```python
from build123d import *

# Parameters (mm, degrees)
SKETCH_1_W                   = 75
SKETCH_1_H                   = 65
EXTRUDE_1_DEPTH              = 7.5
HOLE_WIZARD_M4_1_D           = 4.5
HOLE_WIZARD_M4_1_CBORE_D     = 8
HOLE_WIZARD_M4_1_CBORE_DEPTH = 4.4
HOLE_WIZARD_8_0_8_1_D        = 8
HOLE_WIZARD_1_D              = 4.5
HOLE_WIZARD_1_CBORE_D        = 10
HOLE_WIZARD_1_CBORE_DEPTH    = 7.5
SKETCH_8_R                   = 4
CUT_EXTRUDE_1_DEPTH          = 4.5
CHAMFER_1_SIZE               = 4
SKETCH_9_W                   = 30
SKETCH_9_H                   = 12
CUT_EXTRUDE_2_DEPTH          = 52.841103383
HOLE_WIZARD_M4_1_2_D         = 3.3
FILLET_1_R                   = 3


with BuildPart() as part:
    # 草图1 → 凸台-拉伸1 (new, symmetric)
    with BuildSketch(Plane.XY):
        Rectangle(SKETCH_1_W, SKETCH_1_H)
    extrude(amount=EXTRUDE_1_DEPTH, both=True)

    # Hole Wizard M4 _1 (through all)
    with Locations(Plane.XY.offset(7.5)):
        with Locations((14.5, 1.75), (14.5, -13.75), (30, 1.75), (30, -13.75)):
            CounterBoreHole(HOLE_WIZARD_M4_1_D / 2, HOLE_WIZARD_M4_1_CBORE_D / 2, HOLE_WIZARD_M4_1_CBORE_DEPTH)

    # Ø8.0 (8) 直径孔1 (through all)
    with Locations(Plane.XY.offset(7.5)):
        with Locations((-17.5, 22.5), (-30, -22.5), (-5, -22.5)):
            Hole(HOLE_WIZARD_8_0_8_1_D / 2)

    # 孔1 (through all)
    with Locations(Plane.XY.offset(7.5)):
        with Locations((-17.5, 0), (-17.5, -12.5)):
            CounterBoreHole(HOLE_WIZARD_1_D / 2, HOLE_WIZARD_1_CBORE_D / 2, HOLE_WIZARD_1_CBORE_DEPTH)

    # 草图8 → 切除-拉伸1 (cut)
    with BuildSketch(Plane(origin=(0, 0, -7.5), x_dir=(-1, 0, 0), z_dir=(0, 0, -1))):
        with Locations((17.5, 0)):
            Circle(SKETCH_8_R)
        with Locations((17.5, -12.5)):
            Circle(SKETCH_8_R)
    extrude(amount=-CUT_EXTRUDE_1_DEPTH, mode=Mode.SUBTRACT)

    # 倒角1
    chamfer_1_edges = [part.edges().sort_by_distance(p)[0] for p in [
        (37.5, -32.5, 0),
        (-37.5, -32.5, 0),
        (-37.5, 32.5, 0),
        (37.5, 32.5, 0),
    ]]
    chamfer(chamfer_1_edges, length=CHAMFER_1_SIZE)

    # 草图9 → 切除-拉伸2 (cut, through all)
    with BuildSketch(Plane(origin=(0, 0, -7.5), x_dir=(-1, 0, 0), z_dir=(0, 0, -1))):
        with Locations((-17.5, 13.5)):
            Rectangle(SKETCH_9_W, SKETCH_9_H)
    extrude(amount=-CUT_EXTRUDE_2_DEPTH, mode=Mode.SUBTRACT)

    # Hole Wizard M4 _1 2 (through all)
    with Locations(Plane(origin=(0, 0, -7.5), x_dir=(-1, 0, 0), z_dir=(0, 0, -1))):
        with Locations((-17.5, 24)):
            Hole(HOLE_WIZARD_M4_1_2_D / 2)

    # 圆角1
    fillet_1_edges = [part.edges().sort_by_distance(p)[0] for p in [
        (2.5, 19.5, 0),
        (2.5, 7.5, 0),
        (32.5, 7.5, 0),
        (32.5, 19.5, 0),
    ]]
    fillet(fillet_1_edges, radius=FILLET_1_R)


solid = part.part
```
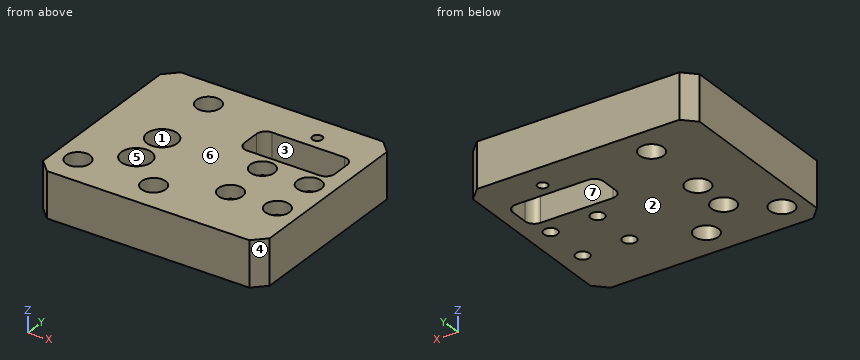
The model under review builds one solid part; all positions refer to its coordinate system, in mm. Face numbers are marked on the shaded views. A direction names the side the tool comes from. Round coordinates to 2 decimals unless told otherwise and drop trailing zeros. Order: outer loops, then holes, each group sorted by start corner. A loop starts at its lowest first (then second) coordinate and runs counter-clockwise, first axis right, second up.
(1) Take a section at B-B, the plane x = -5. State the section outline as (y, z) points, plus the area to 3 significant figures.
Working result:
outline: (-32.5, -7.5) - (-26.5, -7.5) - (-26.5, 7.5) - (-32.5, 7.5) - close; (-18.5, -7.5) - (32.5, -7.5) - (32.5, 7.5) - (-18.5, 7.5) - close
area: 855 mm2
(2) For P1, Ø4, axis at x = 15, y = -13, coming from the +Z side, flat-tipped, find the tip position at first contact; note if it passes through.
Working result:
P1: stops at z = 3.1
(3) Mouldability with a two-part tool opening along X and no side actions: class the marked faces 1, 2, 3 and 4 as released by +X, released by -X, zero draft, split by the parting line, or undercut.
Working result:
face 1: undercut
face 2: zero draft
face 3: undercut
face 4: released by +X
(4) Take a section at A-A, the plane z = -6.5. Count the separate pieces of the cut face and the enclosed holes in it, plus the area to 3 significant figures.
Working result:
separate pieces: 1
enclosed holes: 11
area: 4,170 mm2
(5) Take a section at D-D, the plane x = 30.5. State the section outline as (y, z) points.
Working result:
outline: (-32.5, -7.5) - (-15.94, -7.5) - (-15.94, 3.1) - (-17.72, 3.1) - (-17.72, 7.5) - (-32.5, 7.5) - close; (-11.56, -7.5) - (-0.44, -7.5) - (-0.44, 3.1) - (-2.22, 3.1) - (-2.22, 7.5) - (-9.78, 7.5) - (-9.78, 3.1) - (-11.56, 3.1) - close; (3.94, -7.5) - (7.67, -7.5) - (7.67, 7.5) - (5.72, 7.5) - (5.72, 3.1) - (3.94, 3.1) - close; (19.33, -7.5) - (32.5, -7.5) - (32.5, 7.5) - (19.33, 7.5) - close
(6) Wall thickness on L1, parallel to Y at x = -17.5, z = -1.6; L2, parallel to Y at x = -17.5, z = -4.8; L3, parallel to X at y = 12, z = -1.25: over which ranges is each line inside the solid? List them lowest first.
Working result:
L1: y = -32.5 to -14.75, -10.25 to -2.25, 2.25 to 18.5, 26.5 to 32.5
L2: y = -32.5 to -16.5, -8.5 to -4, 4 to 18.5, 26.5 to 32.5
L3: x = -37.5 to 2.5, 32.5 to 37.5
(7) Take a section at C-C, the plane y = 24. State the section outline as (x, z) points.
Working result:
outline: (-37.5, -7.5) - (-21.21, -7.5) - (-21.21, 7.5) - (-37.5, 7.5) - close; (-13.79, -7.5) - (15.85, -7.5) - (15.85, 7.5) - (-13.79, 7.5) - close; (19.15, -7.5) - (37.5, -7.5) - (37.5, 7.5) - (19.15, 7.5) - close
(8) Tool access review of the marked faces 5, 6 and 7: name each direction out of +Z, -Z, +X, -X, +Y, -Y from which nothing blocks a thin tool from reaching the whole face with its end or side.
Working result:
face 5: +Z
face 6: +Z, +X, -X, +Y, -Y
face 7: +Z, -Z
